The model under review builds one solid part; all positions refer to its coordinate system, in mm. A direction names the side the tool comes from. Round coordinates to 2 decimals unless told otherwise and drop trailing zeros. Loops run counter-clockwise (first coordinate to the right, second up) from the corner with the lowest first, then second, coordinate; pieces in that order, holes last. Notation, with made-up numbers: M 82.5,72.5 L 128.5,72.5 A23 ccw 128.5,100.5 Z; hole C 59.25,-40 d7. An arc over 180 degrees is marked long. Return JSON: item names as keys, results as strings. Group by question number.
Q1. Consider section A-A (y = 32.5). State the section outline as (x, z) points.
Q2. Consider section B-B (x = -73). State the section outline as (y, z) points, and give its area (3 significant figures).
Q3. Consider section C-C (z = -15.25). State the section outline as (x, y) points.
Q4. Draft analysis for pull direction X (two halves, no side actions). For faces 5 (the face through (-155, 3, -12)), 6 (the face through (166, 1, -2)), 7 (the face through (-148.445, 252.979, -12.112)), state which applies: pulls with the +X half, pulls with the -X half, needs draft (parallel to the pull), parting line crosses it, or undercut.
Q5. For faces 1 (the face through (-157, 3, -12)), 2 (the face through (-147.979, -253.445, -12.112)), 3 (the face through (-2, -262, -12)), 4 (the face through (-2, -260, -12)), list the 3-axis set-ups (+Z, -Z, +X, -X, +Y, -Y) from which the entire face can be reached by the end or side of a thin tool; tool diameter is ignored.
Q6. To check wall thickness, follow line 1 along X through (y, z) = (-23, -4.75); line 2 along Y through (x, z) = (116, -12.5); line 3 along Y through (x, z) = (-129, -14.75). State the ranges of each line that lie inside material, in increasing order.
Q7. Clearance check with flat-ended pins moving along their axes: pin 1 Ø1 at (y, z) = (120, -4.5) entering from -X; pin 2 Ø8 at (y, z) = (-94.5, -14) entering from +X; pin 3 Ø8 at (x, z) = (-87.5, -3.5) entering from +Y. State where each tip first meets the part, or that it passes through.
from build123d import *


with BuildPart() as part:
    # Sweep1: sweep along a path in Sketch1
    with BuildLine(Plane.XY) as sweep1_path:
        Line((-127, 260), (127, 260))
        ThreePointArc((127, 260), (146.798989873, 251.798989873), (155, 232))
        Line((155, 232), (155, -232))
        ThreePointArc((155, -232), (146.798989873, -251.798989873), (127, -260))
        Line((127, -260), (-127, -260))
        ThreePointArc((-127, -260), (-146.798989873, -251.798989873), (-155, -232))
        Line((-155, -232), (-155, 232))
        ThreePointArc((-155, 232), (-146.798989873, 251.798989873), (-127, 260))
    # Sketch2 → Sweep1 (sweep)
    with BuildSketch(Plane(origin=(0, 0, 0), x_dir=(1, 0, 0), z_dir=(0, 1, 0))):
        with BuildLine():
            Line((155, 4), (155, 20))
            Line((155, 20), (157, 20))
            Line((157, 20), (157, 4))
            ThreePointArc((157, 4), (157.585786438, 2.585786438), (159, 2))
            Line((159, 2), (172, 2))
            Line((172, 2), (172, 0))
            Line((172, 0), (159, 0))
            ThreePointArc((159, 0), (156.171572875, 1.171572875), (155, 4))
        make_face()
    sweep(path=sweep1_path.line)


solid = part.part
Values:
{
 "1": {"outline": "M -172,-2 L -159,-2 A2 cw -157,-4 L -157,-20 L -155,-20 L -155,-4 A4 ccw -159,0 L -172,0 Z; M 155,-20 L 157,-20 L 157,-4 A2 cw 159,-2 L 172,-2 L 172,0 L 159,0 A4 ccw 155,-4 Z"},
 "2": {"outline": "M -277,-2 L -264,-2 A2 cw -262,-4 L -262,-20 L -260,-20 L -260,-4 A4 ccw -264,0 L -277,0 Z; M 260,-20 L 262,-20 L 262,-4 A2 cw 264,-2 L 277,-2 L 277,0 L 264,0 A4 ccw 260,-4 Z", "area": "135 mm2"},
 "3": {"outline": "M -157,-232 A30 ccw -127,-262 L 127,-262 A30 ccw 157,-232 L 157,232 A30 ccw 127,262 L -127,262 A30 ccw -157,232 Z; hole M -155,-232 A28 ccw -127,-260 L 127,-260 A28 ccw 155,-232 L 155,232 A28 ccw 127,260 L -127,260 A28 ccw -155,232 Z"},
 "4": {"face 5": "undercut", "face 6": "needs draft", "face 7": "pulls with the -X half"},
 "5": {"face 1": "-Z, -X, +Y, -Y", "face 2": "-Z, -X, -Y", "face 3": "-Z, +X, -X, -Y", "face 4": "+Z, -Z"},
 "6": {"line 1": "x = -157 to -155, 155 to 157", "line 2": "y = -262 to -260, 260 to 262", "line 3": "y = -261.93 to -259.93, 259.93 to 261.93"},
 "7": {"pin 1": "stops at x = -157", "pin 2": "stops at x = 157", "pin 3": "stops at y = 277"}
}
